Geometry: final body of the model. Coordinates: model frame, mm. Face numbers are marked on the shaded views. A direction names the side the tool comes from. Coordinates: 2 decimals unless noted, no trailing zeros. Loops run counter-clockwise (first coordinate to the right, second up) from the corner with the lowest first, then second, coordinate; pieces in that order, holes last. Notation, with made-up numbers: (-23.75, 58.5) - (32.25, 58.5) arc R13 ccw to (32.25, 73.5) - close; hole circle Ø4 at (41, -34). An arc over 180 degrees is marked (long way). Return JSON: item names as keys, results as strings.
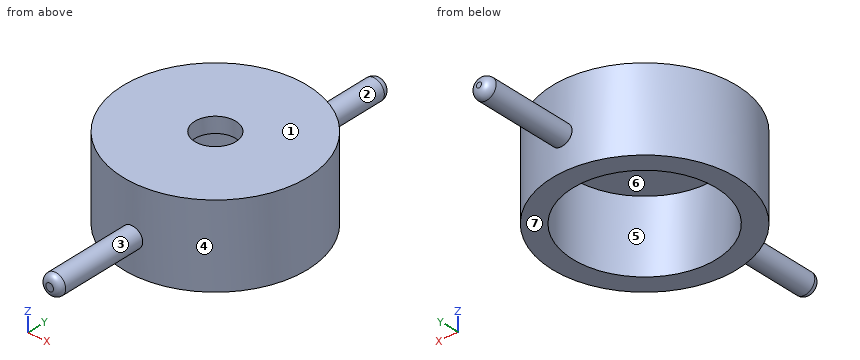
from build123d import *

# Parameters (mm, degrees)
HUB_PROFILE_SKETCH_R       = 36
HUB_72X32_DEPTH            = 32
HANDLE_START               = 35.5
HANDLE_PIN_SKETCH_8_R      = 4
HANDLE_PIN_8_DEPTH         = 36
PIN_END_FILLET_R3_R        = 3
FACE_RECESS_SKETCH_16_R    = 8
FACE_RECESS_16X6_DEPTH     = 6
MIRRORED_PIN_FILLET_R2_5_R = 2.5


with BuildPart() as part:
    # Hub Profile Sketch → Hub Ø72x32 (new body)
    with BuildSketch(Plane.XY):
        Circle(HUB_PROFILE_SKETCH_R)
    extrude(amount=HUB_72X32_DEPTH)

    # Handle Pin Sketch Ø8 → Handle Pin Ø8 (add)
    with BuildSketch(Plane(origin=(0, 0, 0), x_dir=(1, 0, 0), z_dir=(0, 1, 0)).offset(HANDLE_START)):
        with Locations(Location((0, -13, 0), (0, 0, 90))):
            Circle(HANDLE_PIN_SKETCH_8_R)
    handle_pin_8 = extrude(amount=HANDLE_PIN_8_DEPTH)

    # Pin End Fillet R3
    pin_end_fillet_r3_edges = [part.edges().sort_by_distance(p)[0] for p in [
        (0, 71.5, 17),
    ]]
    fillet(pin_end_fillet_r3_edges, radius=PIN_END_FILLET_R3_R)

    # Handle Pin Mirror: Handle Pin Ø8 across plane
    add(handle_pin_8.mirror(Plane.ZX))

    # Revolved Cut Sketch → Revolved Cut (revolve, cut)
    with BuildSketch(Plane(origin=(0, 0, 0), x_dir=(1, 0, 0), z_dir=(0, 1, 0))):
        Polygon((0, -26), (-10, -26), (-10, -28), (-28, -28), (-28, 0), (0, 0), align=None)
    revolve(axis=Axis((0, 0, -9.53547678), (0, 0, 1)), mode=Mode.SUBTRACT)

    # Face Recess Sketch Ø16 → Face Recess Ø16x6 (cut)
    with BuildSketch(Plane.XY.offset(32)):
        Circle(FACE_RECESS_SKETCH_16_R)
    extrude(amount=-FACE_RECESS_16X6_DEPTH, mode=Mode.SUBTRACT)

    # Mirrored Pin Fillet R2.5
    mirrored_pin_fillet_r2_5_edges = [part.edges().sort_by_distance(p)[0] for p in [
        (0, -71.5, 17),
    ]]
    fillet(mirrored_pin_fillet_r2_5_edges, radius=MIRRORED_PIN_FILLET_R2_5_R)


solid = part.part
Item 1: Mould query, pull axis Y, two halves, no side actions, for the marked faces 4, 5, 6 and 7. Classes: +Y half, -Y half, draft (parallel to the pull), parting line (faces both ways), or undercut.
Worked out:
{"face 4": "parting line", "face 5": "undercut", "face 6": "undercut", "face 7": "draft"}
Item 2: Ray query, probe 1 along Y at (x, z) = (0, 27.9); probe 2 along Y at (x, z) = (0, 14); probe 3 along Y at (x, z) = (0, 30). Return the intervals inside material, ascending. Write a range as from..to.
Worked out:
{"probe 1": "-36..-28, -10..-8, 8..10, 28..36", "probe 2": "-71.5..-28, 28..71.5", "probe 3": "-36..-8, 8..36"}
Item 3: Section query D-D, the plane y = -18. Return loops of the section in (x, z).
Worked out:
{"outline": "(-31.18, 0) - (-21.45, 0) - (-21.45, 28) - (21.45, 28) - (21.45, 0) - (31.18, 0) - (31.18, 32) - (-31.18, 32) - close"}
Item 4: First-contact query: pin 1 Ø1 at (y, z) = (27, 17.5) entering from -X; pin 2 Ø5 at (x, y) = (-18.5, -34) entering from -Z; pin 3 Ø2 at (x, z) = (21.5, 12) entering from +Y; pin 4 Ø10 at (x, z) = (-20.5, 12.5) entering from -Y. Flat tips, straight axial feed; report the tip coordinate or a pass-through.
Worked out:
{"pin 1": "x = -24.37", "pin 2": "through", "pin 3": "y = 29.59", "pin 4": "y = -32.49"}
Item 5: Section query A-A, the plane y = 0. Return loops of the section in (x, z).
Worked out:
{"outline": "(-36, 0) - (-28, 0) - (-28, 28) - (-10, 28) - (-10, 26) - (-8, 26) - (-8, 32) - (-36, 32) - close; (8, 26) - (10, 26) - (10, 28) - (28, 28) - (28, 0) - (36, 0) - (36, 32) - (8, 32) - close"}
Item 6: Section query B-B, the plane x = -17. Return loops of the section in (y, z).
Worked out:
{"outline": "(-31.73, 0) - (-22.25, 0) - (-22.25, 28) - (22.25, 28) - (22.25, 0) - (31.73, 0) - (31.73, 32) - (-31.73, 32) - close"}
Item 7: Reachability of the marked faces 1, 2 and 3 from +Z, -Z, +X, -X, +Y, -Y: full face, straight path, thin tool, end or side. Return the list, or none.
Worked out:
{"face 1": "+Z, +X, -X, +Y, -Y", "face 2": "+Y", "face 3": "-Y"}
Item 8: Section query C-C, the plane z = 6. Return loops of the section in (x, y), and give its area (3 significant figures).
Worked out:
{"outline": "circle Ø72 at (0, 0); hole circle Ø56 at (0, 0)", "area": "1,610 mm^2"}
